from build123d import *

# Parameters (mm, degrees)
BOSS_EXTRUDE1_DEPTH = 4
SKETCH2_R           = 2.525
CUT_EXTRUDE1_DEPTH  = 5
BOSS_EXTRUDE2_START = 1.6
SKETCH7_R           = 6
BOSS_EXTRUDE2_DEPTH = 1.6
M4_TAPPED_HOLE1_D   = 3.3
FILLET1_R           = 10


with BuildPart() as part:
    # Sketch1 → Boss-Extrude1 (new body)
    with BuildSketch(Plane.XY):
        with BuildLine():
            Line((3.441458618, -4.914912266), (14.5, 2.828361771))
            Line((14.5, 2.828361771), (25.558541382, -4.914912266))
            ThreePointArc((25.558541382, -4.914912266), (33.914912266, -3.441458618), (32.441458618, 4.914912266))
            Line((32.441458618, 4.914912266), (14.5, 17.477656837))
            Line((14.5, 17.477656837), (-3.441458618, 4.914912266))
            ThreePointArc((-3.441458618, 4.914912266), (-4.914912266, -3.441458618), (3.441458618, -4.914912266))
        make_face()
    extrude(amount=BOSS_EXTRUDE1_DEPTH)

    # Sketch2 → Cut-Extrude1 (cut)
    with BuildSketch(Plane.XY.offset(4)):
        Circle(SKETCH2_R)
    extrude(amount=-CUT_EXTRUDE1_DEPTH, mode=Mode.SUBTRACT)

    # Sketch7 → Boss-Extrude2 (add)
    with BuildSketch(Plane(origin=(0, 0, 0), x_dir=(-1, 0, 0), z_dir=(0, 0, -1)).offset(BOSS_EXTRUDE2_START)):
        with Locations((-29, 0)):
            Circle(SKETCH7_R)
    extrude(amount=-BOSS_EXTRUDE2_DEPTH)

    # M4 Tapped Hole1 (through all)
    with Locations(Plane.XY.offset(4)):
        with Locations((29, 0)):
            Hole(M4_TAPPED_HOLE1_D / 2)

    # Fillet1
    fillet1_edges = [part.edges().sort_by_distance(p)[0] for p in [
        (14.5, 17.477656837, 2),
        (14.5, 2.828361771, 2),
    ]]
    fillet(fillet1_edges, radius=FILLET1_R)


solid = part.part
CAD build for the part. Positions are in the model's coordinates, mm. A direction names the side the tool comes from. Round coordinates to 2 decimals unless told otherwise and drop trailing zeros. Loops run counter-clockwise (first coordinate to the right, second up) from the corner with the lowest first, then second, coordinate; pieces in that order, holes last. Notation, with made-up numbers: M 44,22.5 L 80,22.5 A25 cw 80,60.5 Z; hole C 22,53 d8. An arc over 180 degrees is marked long. One line per question, with ' | ' between items. Start each with the question number.
Item 1: Wall check: line 1 (X direction, y = -2.25, z = 3.15); line 2 (Y direction, x = 29, z = -0.3); line 3 (X direction, y = 1.5, z = 1.6). Give the ranges that are in metal, low to high.
Item 2: Pin check, flat tips, straight feed: pin 1 Ø8 at (x, y) = (21, 8) entering from -Z; pin 2 Ø3 at (y, z) = (0.5, 3.5) entering from -X. Stop position of each tip, or through.
Item 3: Which spindle directions (+Z, -Z, +X, -X, +Y, -Y) get a long thin tool onto all of the face, cutting with end or side? Do faces 4 (the flat face through (2.75, 9.25, 1.97)), 5 (the flat face through (22.86, -3.025, 1.972)). Say none if no direction does.
Item 4: Two-plate mould, pull along X, no slides. Class faces 1 (the cylindrical face through (14.41, 15.27, 2.03)), 2 (the flat face through (14, 5, 4)), 3 (the cylindrical face through (14.59, 0.62, 2.03)): pulls with the +X half, pulls with the -X half, needs draft (parallel to the pull), parting line crosses it, or undercut.
Item 5: Cut at D-D, the plane z = -0.5. Write the cut outline in (x, y).
Item 6: Cut at B-B, the plane x = 0. Write the cut outline in (y, z) (3 decimals).
Item 7: Cut at A-A, the plane y = -0.5. Write the cut outline in (x, z) (3 decimals), plus the area to 3 significant figures.
Item 8: Cut at C-C, the plane y = -3. Write the cut outline in (x, z), plus the area to 3 significant figures.
Responses:
1) line 1: x = -5.56 to -1.15, 1.15 to 7.25, 21.75 to 34.56 | line 2: y = -6 to -1.65, 1.65 to 6 | line 3: x = -5.81 to -2.03, 2.03 to 28.31, 29.69 to 34.81
2) pin 1: stops at z = 0 | pin 2: stops at x = -6
3) face 4: +Z, -Z, -X, +Y | face 5: +Z, -Z, -Y
4) face 1: parting line crosses it | face 2: needs draft | face 3: undercut
5) outline: C 29,0 d12; hole C 29,0 d3.3
6) outline: M -6,0 L -2.525,0 L -2.525,4 L -6,4 Z; M 2.525,0 L 7.325,0 L 7.325,4 L 2.525,4 Z
7) outline: M -5.979,0 L -2.475,0 L -2.475,4 L -5.979,4 Z; M 2.475,0 L 9.9,0 L 9.9,4 L 2.475,4 Z; M 19.1,0 L 23.021,0 L 23.021,-1.6 L 27.428,-1.6 L 27.428,4 L 19.1,4 Z; M 30.572,-1.6 L 34.979,-1.6 L 34.979,4 L 30.572,4 Z | area: 109 mm²
8) outline: M -5.2,0 L 6.18,0 L 6.18,4 L -5.2,4 Z; M 22.82,0 L 23.8,0 L 23.8,-1.6 L 34.2,-1.6 L 34.2,4 L 22.82,4 Z | area: 108 mm²
